For this review, take the finished solid that the model builds, in its own axes (mm). A direction names the side the tool comes from. Round coordinates to 2 decimals unless told otherwise and drop trailing zeros. Order: outer loops, then holes, each group sorted by start corner. A loop starts at its lowest first (then second) coordinate and runs counter-clockwise, first axis right, second up. Notation, with made-up numbers: M -1,14.25 L 14,14.25 A24 cw 14,39.25 Z; hole C -29.75,51.25 d1. An arc over 180 degrees is marked long. Answer as a JSON object with one key per item and string values.
from build123d import *

# Parameters (mm, degrees)
BOSS_EXTRUDE1_DEPTH   = 460
SKETCH2_W             = 400
SKETCH2_H             = 80
CUT_EXTRUDE1_DEPTH    = 50
SKETCH3_R             = 16
CUT_EXTRUDE2_DEPTH    = 475.523181731
M6_TAPPED_HOLE1_D     = 5
M6_TAPPED_HOLE1_DEPTH = 17
M6_TAPPED_HOLE1_TIP   = 1.502151548
M6_TAPPED_HOLE2_D     = 5
M6_TAPPED_HOLE2_DEPTH = 17
M6_TAPPED_HOLE2_TIP   = 1.502151548


with BuildPart() as part:
    # Sketch1 → Boss-Extrude1 (new body)
    with BuildSketch(Plane(origin=(0, 0, 0), x_dir=(0, 0, -1), z_dir=(1, 0, 0))):
        Polygon((-104, 12.5), (-47.702939672, 12.5), (-46.297660938, 11.076907706), (-44.163022497, 13.184825808), (-45.568301231, 14.607918102), (-70, 49.5), (-70, 52.5), (-5, 52.5), (-5, 49.916740154), (5, 49.916740154), (5, 52.5), (70, 52.5), (70, 49.5), (45.568301231, 14.607918102), (44.163022497, 13.184825808), (46.297660938, 11.076907706), (47.702939672, 12.5), (104, 12.5), (104, -12.5), (-104, -12.5), align=None)
    extrude(amount=BOSS_EXTRUDE1_DEPTH)

    # Sketch2 → Cut-Extrude1 (cut)
    with BuildSketch(Plane(origin=(0, 52.5, 0), x_dir=(1, 0, 0), z_dir=(0, 1, 0))):
        with Locations((230, 0)):
            Rectangle(SKETCH2_W, SKETCH2_H)
    extrude(amount=-CUT_EXTRUDE1_DEPTH, mode=Mode.SUBTRACT)

    # Sketch3 → Cut-Extrude2 (cut, through all)
    with BuildSketch(Plane(origin=(460, 0, 0), x_dir=(0, 0, -1), z_dir=(1, 0, 0))):
        with Locations((0, 30.5)):
            Circle(SKETCH3_R)
    extrude(amount=-CUT_EXTRUDE2_DEPTH, mode=Mode.SUBTRACT)

    # M6 Tapped Hole1
    with Locations(Plane(origin=(460, 0, 0), x_dir=(0, 0, -1), z_dir=(1, 0, 0))):
        with Locations((-20.5, 30.5), (20.5, 30.5)):
            Hole(M6_TAPPED_HOLE1_D / 2, depth=M6_TAPPED_HOLE1_DEPTH)
            with Locations((0, 0, -(M6_TAPPED_HOLE1_DEPTH + M6_TAPPED_HOLE1_TIP / 2))):  # 118° drill point
                Cone(0, M6_TAPPED_HOLE1_D / 2, M6_TAPPED_HOLE1_TIP, mode=Mode.SUBTRACT)

    # M6 Tapped Hole2
    with Locations(Plane.ZY):
        with Locations((17.453686729, 19.747381031), (-17.453687008, 41.252618969)):
            Hole(M6_TAPPED_HOLE2_D / 2, depth=M6_TAPPED_HOLE2_DEPTH)
            with Locations((0, 0, -(M6_TAPPED_HOLE2_DEPTH + M6_TAPPED_HOLE2_TIP / 2))):  # 118° drill point
                Cone(0, M6_TAPPED_HOLE2_D / 2, M6_TAPPED_HOLE2_TIP, mode=Mode.SUBTRACT)


solid = part.part
1) Insertion check: P1, Ø3.5, axis at x = 319, y = 51, coming from the -Z side; P2, Ø2, axis at x = 443, y = 51.5, coming from the +Z side; P3, Ø1.5, axis at x = 114, y = 43, coming from the +Z side. Each pin has a flat end and moves straight along its axis. Give the tip position at first contact, or say it passes through.
Geometry check:
{"P1": "stops at z = -70", "P2": "stops at z = 70", "P3": "stops at z = 65.97"}
2) Mouldability with a two-part tool opening along Y and no side actions: class faces 4 (the flat face through (15, 49.917, 0)), 5 (the flat face through (227, 12.5, 76)), 6 (the flat face through (227, 28, -40)) as +Y half, -Y half, draft (parallel to the pull), parting line (faces both ways), or undercut.
Geometry check:
{"face 4": "+Y half", "face 5": "undercut", "face 6": "draft"}
3) Add section B-B on x = 207. State the section outline as (y, z) points, and give its area (3 significant figures).
Geometry check:
{"outline": "M -12.5,-104 L 12.5,-104 L 12.5,-47.7 L 11.08,-46.3 L 13.18,-44.16 L 14.61,-45.57 L 49.5,-70 L 52.5,-70 L 52.5,-40 L 2.5,-40 L 2.5,40 L 52.5,40 L 52.5,70 L 49.5,70 L 14.61,45.57 L 13.18,44.16 L 11.08,46.3 L 12.5,47.7 L 12.5,104 L -12.5,104 Z", "area": "5,840 mm²"}
4) Add section D-D on z = 83. State the section outline as (x, y) points, and give its area (3 significant figures).
Geometry check:
{"outline": "M 0,-12.5 L 460,-12.5 L 460,12.5 L 0,12.5 Z", "area": "11,500 mm²"}
5) For L1, parallel to Y at x = 448.25, z = 20.5; L2, parallel to Y at x = 9.75, z = 0; L3, parallel to Z at x = 450, y = 30, list the stretches that pass through material, from the lowest coordinate up.
Geometry check:
{"L1": "y = -12.5 to 28, 33 to 52.5", "L2": "y = -12.5 to 14.5, 46.5 to 49.92", "L3": "z = -56.35 to -22.95, -18.05 to -15.99, 15.99 to 18.05, 22.95 to 56.35"}
6) Machinability: for faces 1 (the flat face through (30, 17, 9)), 2 (the flat face through (445, 49.917, 0)), 3 (the flat face through (226.78, 32.298, -57.955)), which of the approach directions +Z, -Z, +X, -X, +Y, -Y give a long, thin tool a straight path to every point of the face, cutting with its end or side? Answer none if there is none.
Geometry check:
{"face 1": "+Y", "face 2": "+X, -X, +Y", "face 3": "-Z, +X, -X"}
7) Add section C-C on z = 58. State the section outline as (x, y) points.
Geometry check:
{"outline": "M 0,-12.5 L 460,-12.5 L 460,12.5 L 0,12.5 Z; M 0,32.36 L 460,32.36 L 460,52.5 L 0,52.5 Z"}
8) Add section A-A on z = 0. State the section outline as (x, y) points.
Geometry check:
{"outline": "M 0,-12.5 L 460,-12.5 L 460,14.5 L 430,14.5 L 430,2.5 L 30,2.5 L 30,14.5 L 0,14.5 Z; M 0,46.5 L 30,46.5 L 30,49.92 L 0,49.92 Z; M 430,46.5 L 460,46.5 L 460,49.92 L 430,49.92 Z"}
